```python
from build123d import *

# Parameters (mm, degrees)
SKETCH_1_W          = 200
SKETCH_1_H          = 160
EXTRUDE_1_DEPTH     = 12
CUT_EXTRUDE_1_DEPTH = 12


with BuildPart() as part:
    # 草图1 → 凸台-拉伸1 (new body)
    with BuildSketch(Plane.XY):
        Rectangle(SKETCH_1_W, SKETCH_1_H)
    extrude(amount=EXTRUDE_1_DEPTH)

    # 草图2 → 切除-拉伸1 (cut)
    with BuildSketch(Plane.XY.offset(12)):
        Polygon((-100, 40), (-40, -80), (-100, -80), align=None)
        Polygon((-21, -80), (0, 40), (100, 40), (100, -80), align=None)
    extrude(amount=-CUT_EXTRUDE_1_DEPTH, mode=Mode.SUBTRACT)


solid = part.part
```
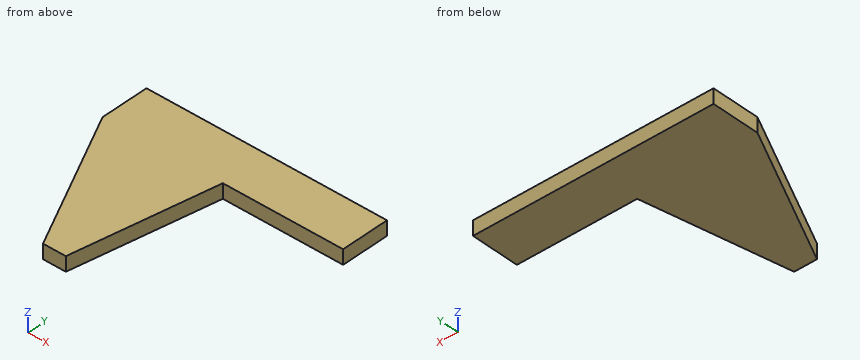
Part model, mm, in its own coordinate system. Give positions to 0.01 mm unless a question says otherwise; leave off trailing zeros. Order: outer loops, then holes, each group sorted by start corner. A loop starts at its lowest first (then second) coordinate and runs counter-clockwise, first axis right, second up. Notation, with made-up numbers: (-2.5, 74) - (11.5, 74) arc R35 ccw to (11.5, 106) - close; hole circle Ø8 at (60, -31.75). An arc over 180 degrees is marked (long way). Use one line per item in the form item = value.
Item 1: Slice it at B-B on y = 36. Give the cut face in (x, z).
Solution:
outline = (-98, 0) - (-0.7, 0) - (-0.7, 12) - (-98, 12) - close
Item 2: Slice it at C-C on x = -65. Give the cut face in (y, z).
Solution:
outline = (-30, 0) - (80, 0) - (80, 12) - (-30, 12) - close
Item 3: Probe probe 1 along Y at (x, z) = (69.5, 2.25); probe 2 along Y at (x, z) = (-56.5, 2.25); probe 3 along X at (y, z) = (30, 5). List the from-to ranges inside material, lowest first. Write a range as from..to.
Solution:
probe_1 = 40..80
probe_2 = -47..80
probe_3 = -95..-1.75
Item 4: Slice it at A-A on z = 3. Give the cut face in (x, y).
Solution:
outline = (-100, 40) - (-40, -80) - (-21, -80) - (0, 40) - (100, 40) - (100, 80) - (-100, 80) - close
Item 5: Pin check, flat tips, straight feed: pin 1 Ø1 at (y, z) = (-20, 5.5) entering from +X; pin 2 Ø6 at (x, z) = (42.5, 8.5) entering from -Y; pin 3 Ø5 at (x, z) = (-65, 4) entering from -Y. Stop position of each tip, or through.
Solution:
pin_1 = -10.41
pin_2 = 40
pin_3 = -35
